Input: part model. Units: mm. Frame: model coordinates. A direction names the side the tool comes from. Give positions to 0.01 mm unless a question says otherwise; leave off trailing zeros. Loops run counter-clockwise (first coordinate to the right, second up) from the corner with the lowest first, then second, coordinate; pieces in that order, holes last. Notation, with made-up numbers: M 18,-27.5 L 75,-27.5 A15 cw 75,-18.5 Z; hole C -17,13 d7. An arc over 180 degrees is marked long. Answer as a JSON object with one key per item and string values. Group by question number.
1) Section query A-A on y = 27.5. Return loops of the section in (x, z), plus the area to 3 significant figures.
2) Draft query along X for faces 1 (the flat face through (-35, -17, -22)), 2 (the conical face through (-48.153, 39.84, -0.819)), 3 (the flat face through (0, -7, 0)). Return one class per face: +X half, -X half, draft (parallel to the pull), parting line (faces both ways), or undercut.
3) Access query for faces 4 (the flat face through (0, 140, 0)), 5 (the flat face through (13.2, 44, 24.3)), 6 (the cylindrical face through (25.861, -3.944, -33.727)). Directions: +Z, -Z, +X, -X, +Y, -Y. A direction counts if a zero-diameter tool reaches every point of the face in a straight line with its end or side. Return the directions, or none.
4) First-contact query: P1, Ø10, axis at y = 19.5, z = -32, coming from the +X side; P2, Ø2, axis at x = 28.5, y = 68, coming from the -Z side; P3, Ø1, axis at x = 21.5, y = -36.5, coming from the -Z side. Flat tips, straight axial feed; report the tip coordinate or a pass-through.
5) Section query B-B on y = -26. Return loops of the section in (x, z), plus the area to 3 significant figures.
6) Ray query, L1, parallel to X at y = -35, z = 0; L2, parallel to Y at x = -18, z = -21.5; L3, parallel to Y at x = -14.5, z = 38.5. Return the intervals inside material, ascending.
7) Section query C-C on y = 102. Return loops of the section in (x, z).
from build123d import *

# Parameters (mm, degrees)
SKETCH1_R           = 49
BOSS_EXTRUDE1_DEPTH = 40
SKETCH2_R           = 30
BOSS_EXTRUDE2_DEPTH = 100
SKETCH3_R           = 42.5
BOSS_EXTRUDE3_DEPTH = 9
SKETCH4_R           = 41
BOSS_EXTRUDE4_DEPTH = 8
SKETCH5_R           = 42.5
BOSS_EXTRUDE5_DEPTH = 40
CHAMFER1_SIZE       = 1
SKETCH6_W           = 154
SKETCH6_H           = 25
CUT_EXTRUDE1_DEPTH  = 25
CUT_EXTRUDE4_DEPTH  = 157.211395231
CUT_EXTRUDE5_DEPTH  = 157.211395231
SKETCH10_R          = 60.311534853
SKETCH10_R_2        = 27.5
CUT_EXTRUDE6_DEPTH  = 4
SKETCH13_R          = 25
CUT_EXTRUDE7_DEPTH  = 50


with BuildPart() as part:
    # Sketch1 → Boss-Extrude1 (new body)
    with BuildSketch(Plane(origin=(0, 0, 0), x_dir=(1, 0, 0), z_dir=(0, 1, 0))):
        with Locations(Location((0, 0, 0), (0, 0, 270))):
            Circle(SKETCH1_R)
    extrude(amount=BOSS_EXTRUDE1_DEPTH)

    # Sketch2 → Boss-Extrude2 (add)
    with BuildSketch(Plane(origin=(0, 40, 0), x_dir=(1, 0, 0), z_dir=(0, 1, 0))):
        with Locations(Location((0, 0, 0), (0, 0, 270))):
            Circle(SKETCH2_R)
    extrude(amount=BOSS_EXTRUDE2_DEPTH)

    # Sketch3 → Boss-Extrude3 (add)
    with BuildSketch(Plane.XZ):
        with Locations(Location((0, 0, 0), (0, 0, 90))):
            Circle(SKETCH3_R)
    extrude(amount=BOSS_EXTRUDE3_DEPTH)

    # Sketch4 → Boss-Extrude4 (add)
    with BuildSketch(Plane.XZ.offset(9)):
        with Locations(Location((0, 0, 0), (0, 0, 270))):
            Circle(SKETCH4_R)
    extrude(amount=BOSS_EXTRUDE4_DEPTH)

    # Sketch5 → Boss-Extrude5 (add)
    with BuildSketch(Plane.XZ.offset(17)):
        with Locations(Location((0, 0, 0), (0, 0, 90))):
            Circle(SKETCH5_R)
    extrude(amount=BOSS_EXTRUDE5_DEPTH)

    # Chamfer1
    chamfer1_edges = [part.edges().sort_by_distance(p)[0] for p in [
        (0, -9, -42.5),
        (0, -57, -42.5),
        (0, 40, -49),
        (0, 140, -30),
    ]]
    chamfer(chamfer1_edges, length=CHAMFER1_SIZE)

    # Sketch6 → Cut-Extrude1 (cut)
    with BuildSketch(Plane(origin=(0, 40, 0), x_dir=(1, 0, 0), z_dir=(0, 1, 0))):
        with Locations((0, 57.5)):
            Rectangle(SKETCH6_W, SKETCH6_H)
        with Locations((0, -57.5)):
            Rectangle(SKETCH6_W, SKETCH6_H)
    extrude(amount=-CUT_EXTRUDE1_DEPTH, mode=Mode.SUBTRACT)

    # Sketch 9_2 → Cut-Extrude4 (cut, through all)
    with BuildSketch(Plane(origin=(0, 0, 0), x_dir=(0, 0, -1), z_dir=(1, 0, 0))):
        Polygon((-45, 15), (-52.848399212, 15), (-52.983105111, 7.016894889), align=None)
        Polygon((45, 15), (54.94145121, 15), (54.048754667, 5.951245333), align=None)
    extrude(amount=-CUT_EXTRUDE4_DEPTH, mode=Mode.SUBTRACT)

    # Sketch 9_2 2 → Cut-Extrude5 (cut, through all)
    with BuildSketch(Plane(origin=(0, 0, 0), x_dir=(0, 0, -1), z_dir=(1, 0, 0))):
        Polygon((-45, 15), (-52.848399212, 15), (-52.983105111, 7.016894889), align=None)
        Polygon((45, 15), (54.94145121, 15), (54.048754667, 5.951245333), align=None)
    extrude(amount=CUT_EXTRUDE5_DEPTH, mode=Mode.SUBTRACT)

    # Sketch10 → Cut-Extrude6 (cut)
    with BuildSketch(Plane(origin=(0, 40, 0), x_dir=(1, 0, 0), z_dir=(0, 1, 0))):
        Circle(SKETCH10_R)
        with Locations(Location((0, 0, 0), (0, 0, 270))):
            Circle(SKETCH10_R_2, mode=Mode.SUBTRACT)
    extrude(amount=CUT_EXTRUDE6_DEPTH, mode=Mode.SUBTRACT)

    # Sketch13 → Cut-Extrude7 (cut)
    with BuildSketch(Plane.XZ.offset(57)):
        with Locations(Location((0, 0, 0), (0, 0, 270))):
            Circle(SKETCH13_R)
    extrude(amount=-CUT_EXTRUDE7_DEPTH, mode=Mode.SUBTRACT)


solid = part.part
Output:
{
 "1": {"outline": "M -19.39,-45 L 19.39,-45 A49 ccw 19.39,45 L -19.39,45 A49 ccw Z", "area": "7,330 mm^2"},
 "2": {"face 1": "draft", "face 2": "-X half", "face 3": "undercut"},
 "3": {"face 4": "+Z, -Z, +X, -X, +Y", "face 5": "none", "face 6": "-Y"},
 "4": {"P1": "stops at x = 40.89", "P2": "stops at z = -11.99", "P3": "stops at z = -36.95"},
 "5": {"outline": "C 0,0 d85; hole C 0,0 d50", "area": "3,710 mm^2"},
 "6": {"L1": "x = -42.5 to -25, 25 to 42.5", "L2": "y = -57 to 40, 44 to 140", "L3": "y = -57 to -17, -9 to 40"},
 "7": {"outline": "C 0,0 d60"}
}
